For this review, take the finished solid that the model builds, in its own axes (mm). A direction names the side the tool comes from. Give positions to 0.01 mm unless a question says otherwise; leave off trailing zeros. Order: outer loops, then holes, each group sorted by start corner. A loop starts at its lowest first (then second) coordinate and runs counter-clockwise, first axis right, second up. Notation, with made-up numbers: (-29, 11) - (-18, 11) arc R27 ccw to (-18, 42) - close; hole circle Ø5 at (4, -12). An arc over 180 degrees is marked (long way). Use a Markdown table: item, result. Add a question column.
1) We need section D-D on y = 13. Write out the cut boundary in (x, z).
2) Wall thickness on L1, parallel to Z at x = 35, y = 23; L2, parallel to Y at x = 118, z = 74; L3, parallel to Y at x = 25, z = 6.5: over which ranges is each line inside the solid? List them lowest first.
3) We need section A-A on x = 64.5. Write out the cut boundary in (y, z), then the cut area to 3 significant figures.
4) We need section B-B on x = 25. Write out the cut boundary in (y, z), then the cut area to 3 significant figures.
5) Mouldability with a two-part tool opening along Z and no side actions: class faces 1 (the face through (62, 19, 0)), 2 (the face through (125, 19, 47)), 3 (the face through (51, 30, 29)) as released by +Z, released by -Z, zero draft, split by the parting line, or undercut.
6) Clearance check with flat-ended pins moving along their axes: P1, Ø3, axis at x = 64.5, z = 19, coming from the -Y side; P2, Ø10, axis at y = 6, z = 72.5, coming from the -X side; P3, Ø21, axis at x = 25, y = 13, coming from the +Z side. State where each tip first meets the part, or that it passes through.
7) Machinability: for faces 4 (the face through (49, 11, 10)), 5 (the face through (51, 30, 45)), 6 (the face through (49, 30, 55)), 7 (the face through (113, 19, 93)), which of the approach directions +Z, -Z, +X, -X, +Y, -Y give a long, thin tool a straight path to every point of the face, cutting with its end or side? Answer none if there is none.
8) We need section C-C on z = 37.5. Write out the cut boundary in (x, y), then the cut area to 3 significant figures.
```python
from build123d import *

# Parameters (mm, degrees)
BASE_PLATE_SKETCH_W   = 125
BASE_PLATE_SKETCH_H   = 38
BASE_PLATE_DEPTH      = 10
HINGE_LUG_DEPTH       = 25
LUG_BORE_19_SKETCH_R  = 9.5
LUG_BORE_19_DEPTH     = 25
ARM_SKETCH_W          = 100
ARM_SKETCH_H          = 45
ARM_DEPTH             = 16
SLOT_70X16_SKETCH_W   = 70
SLOT_70X16_SKETCH_H   = 16
SLOT_70X16_DEPTH      = 16
CORNER_NOTCH_SKETCH_R = 6.5
CORNER_NOTCH_DEPTH    = 10


with BuildPart() as part:
    # Base Plate Sketch → Base Plate (new body)
    with BuildSketch(Plane.XY):
        with Locations((62.5, 19)):
            Rectangle(BASE_PLATE_SKETCH_W, BASE_PLATE_SKETCH_H)
    extrude(amount=BASE_PLATE_DEPTH)

    # Hinge Lug Sketch → Hinge Lug (add)
    with BuildSketch(Plane(origin=(125, 0, 0), x_dir=(0, 0, -1), z_dir=(1, 0, 0))):
        with BuildLine():
            Line((-10, 38), (-74, 38))
            ThreePointArc((-74, 38), (-93, 19), (-74, 0))
            Line((-74, 0), (-10, 0))
            Line((-10, 0), (-10, 38))
        make_face()
    extrude(amount=-HINGE_LUG_DEPTH)

    # Lug Bore Ø19 Sketch → Lug Bore Ø19 (cut)
    with BuildSketch(Plane(origin=(125, 0, 0), x_dir=(0, 0, -1), z_dir=(1, 0, 0))):
        with Locations((-74, 19)):
            Circle(LUG_BORE_19_SKETCH_R)
    extrude(amount=-LUG_BORE_19_DEPTH, mode=Mode.SUBTRACT)

    # Arm Sketch → Arm (add)
    with BuildSketch(Plane(origin=(0, 38, 0), x_dir=(1, 0, 0), z_dir=(0, 1, 0))):
        with Locations((50, -32.5)):
            Rectangle(ARM_SKETCH_W, ARM_SKETCH_H)
    extrude(amount=-ARM_DEPTH)

    # Slot 70x16 Sketch → Slot 70x16 (cut)
    with BuildSketch(Plane(origin=(0, 38, 0), x_dir=(1, 0, 0), z_dir=(0, 1, 0))):
        with Locations((51, -37)):
            Rectangle(SLOT_70X16_SKETCH_W, SLOT_70X16_SKETCH_H)
    extrude(amount=-SLOT_70X16_DEPTH, mode=Mode.SUBTRACT)

    # Corner Notch Sketch → Corner Notch (cut)
    with BuildSketch(Plane.XY.offset(10)):
        with Locations((25, 13)):
            Circle(CORNER_NOTCH_SKETCH_R)
        with Locations((75, 13)):
            Circle(CORNER_NOTCH_SKETCH_R)
    extrude(amount=-CORNER_NOTCH_DEPTH, mode=Mode.SUBTRACT)


solid = part.part
```
Checked values:
| question | item | result |
|---|---|---|
| 1 | outline | (0, 0) - (18.5, 0) - (18.5, 10) - (0, 10) - close; (31.5, 0) - (68.5, 0) - (68.5, 10) - (31.5, 10) - close; (81.5, 0) - (125, 0) - (125, 66.63) - (100, 66.63) - (100, 10) - (81.5, 10) - close; (100, 81.37) - (125, 81.37) - (125, 92.03) - (100, 92.03) - close |
| 2 | L1 | 0 to 29, 45 to 55 |
| 2 | L2 | 0 to 9.5, 28.5 to 38 |
| 2 | L3 | 0 to 6.5, 19.5 to 38 |
| 3 | outline | (0, 0) - (38, 0) - (38, 29) - (22, 29) - (22, 10) - (0, 10) - close; (22, 45) - (38, 45) - (38, 55) - (22, 55) - close |
| 3 | area | 844 mm² |
| 4 | outline | (0, 0) - (6.5, 0) - (6.5, 10) - (0, 10) - close; (19.5, 0) - (38, 0) - (38, 29) - (22, 29) - (22, 10) - (19.5, 10) - close; (22, 45) - (38, 45) - (38, 55) - (22, 55) - close |
| 4 | area | 714 mm² |
| 5 | face 1 | released by -Z |
| 5 | face 2 | zero draft |
| 5 | face 3 | undercut |
| 6 | P1 | y = 22 |
| 6 | P2 | x = 100 |
| 6 | P3 | z = 55 |
| 7 | face 4 | +Z, -X, -Y |
| 7 | face 5 | +Y, -Y |
| 7 | face 6 | +Z, -X, +Y, -Y |
| 7 | face 7 | +Z, +X, -X |
| 8 | outline | (0, 22) - (16, 22) - (16, 38) - (0, 38) - close; (86, 22) - (100, 22) - (100, 0) - (125, 0) - (125, 38) - (86, 38) - close |
| 8 | area | 1,430 mm² |
